Part model, mm, in its own coordinate system. A direction names the side the tool comes from. Round coordinates to 2 decimals unless told otherwise and drop trailing zeros. Loops run counter-clockwise (first coordinate to the right, second up) from the corner with the lowest first, then second, coordinate; pieces in that order, holes last. Notation, with made-up numbers: (27, 40) - (76, 40) arc R34 ccw to (76, 75) - close; hole circle Ø7 at (87, -3). An arc over 180 degrees is marked (long way). Write each question's results on one line, items separated by ' | '. Start each with the question number.
(1) Tool access for faces 1 (the face through (-57, 32, 1)), 2 (the face through (-54, 19, 1)): list every direction of +Z, -Z, +X, -X, +Y, -Y with a clear straight run to the whole face (end or side of a thin tool).
(2) Flat gauge pin, fed straight in: P1, Ø3, axis at x = 33.5, z = -16.5, coming from the +Y side. Where does the tip first touch, or does it go through?
(3) Cut at A-A, the plane y = 9. List the corners of the cut face in (x, z), then the cut area to 3 significant figures.
(4) Mould opens along X. For faces 3 (the face through (54, 19, 1)), 4 (the face through (0, 4, -45)), 5 (the face through (-60, 16, 1)) say: released by +X, released by -X, zero draft, split by the parting line, or undercut.
(5) Cut at C-C, the plane x = 38.5. List the corners of the cut face in (y, z), then the cut area to 3 significant figures.
(6) Drill centre lines: L1, parallel to X at y = 10.5, z = -33.5; L2, parallel to Y at x = 50, z = 11.5. Where is each one in solid material? Low to high.
(7) Cut at B-B, the plane z = 12. List the corners of the cut face in (x, y), then the cut area to 3 significant figures.
from build123d import *

# Parameters (mm, degrees)
EXTRUDE_1_DEPTH = 45


with BuildPart() as part:
    # 草图1 → 凸台-拉伸1 (new, symmetric)
    with BuildSketch(Plane.XY):
        Polygon((-60, 0), (60, 0), (60, 32), (54, 32), (54, 6), (-54, 6), (-54, 32), (-60, 32), align=None)
    extrude(amount=EXTRUDE_1_DEPTH, both=True)


solid = part.part
A:
1) face 1: +Z, -Z, +X, -X, +Y | face 2: +Z, -Z, +Y
2) P1: y = 6
3) outline: (-60, -45) - (-54, -45) - (-54, 45) - (-60, 45) - close; (54, -45) - (60, -45) - (60, 45) - (54, 45) - close | area: 1,080 mm2
4) face 3: undercut | face 4: zero draft | face 5: released by -X
5) outline: (0, -45) - (6, -45) - (6, 45) - (0, 45) - close | area: 540 mm2
6) L1: -60 to -54, 54 to 60 | L2: 0 to 6
7) outline: (-60, 0) - (60, 0) - (60, 32) - (54, 32) - (54, 6) - (-54, 6) - (-54, 32) - (-60, 32) - close | area: 1,030 mm2
